Model file for the job. Use its own axes, mm. Coordinates: 2 decimals unless noted, no trailing zeros. Loops run counter-clockwise (first coordinate to the right, second up) from the corner with the lowest first, then second, coordinate; pieces in that order, holes last. Notation, with made-up numbers: M 33.25,14 L 79.25,14 A18 ccw 79.25,44 Z; hole C 74.5,34 d6. An arc over 180 degrees is marked long. One line per question, with ' | ' between items. Start each with the question number.
```python
from build123d import *

# Parameters (mm, degrees)
SKETCH_1_W                   = 20
SKETCH_1_H                   = 220
EXTRUDE_1_DEPTH              = 17.5
HOLE_WIZARD_M8_1_D           = 9
HOLE_WIZARD_M8_1_CBORE_D     = 15
HOLE_WIZARD_M8_1_CBORE_DEPTH = 8.6
HOLE_WIZARD_M8_1_2_D         = 6.8
HOLE_WIZARD_M8_1_2_DEPTH     = 19.75
HOLE_WIZARD_M8_1_2_TIP       = 2.042926105
CHAMFER_1_SIZE               = 1


with BuildPart() as part:
    # 草图1 → 凸台-拉伸1 (new, symmetric)
    with BuildSketch(Plane.XY):
        Rectangle(SKETCH_1_W, SKETCH_1_H)
    extrude(amount=EXTRUDE_1_DEPTH, both=True)

    # Hole Wizard M8 _1 (through all)
    with Locations(Plane.XY.offset(17.5)):
        with Locations((0, 100), (0, 0), (0, -100)):
            CounterBoreHole(HOLE_WIZARD_M8_1_D / 2, HOLE_WIZARD_M8_1_CBORE_D / 2, HOLE_WIZARD_M8_1_CBORE_DEPTH)

    # Hole Wizard M8 _1 2
    with Locations(Plane.XY.offset(17.5)):
        with Locations((0, 80), (0, -80)):
            Hole(HOLE_WIZARD_M8_1_2_D / 2, depth=HOLE_WIZARD_M8_1_2_DEPTH)
            with Locations((0, 0, -(HOLE_WIZARD_M8_1_2_DEPTH + HOLE_WIZARD_M8_1_2_TIP / 2))):  # 118° drill point
                Cone(0, HOLE_WIZARD_M8_1_2_D / 2, HOLE_WIZARD_M8_1_2_TIP, mode=Mode.SUBTRACT)

    # 倒角1
    chamfer_1_edges = [part.edges().sort_by_distance(p)[0] for p in [
        (10, -110, 0),
        (-10, -110, 0),
        (-10, 110, 0),
        (10, 110, 0),
    ]]
    chamfer(chamfer_1_edges, length=CHAMFER_1_SIZE)


solid = part.part
```
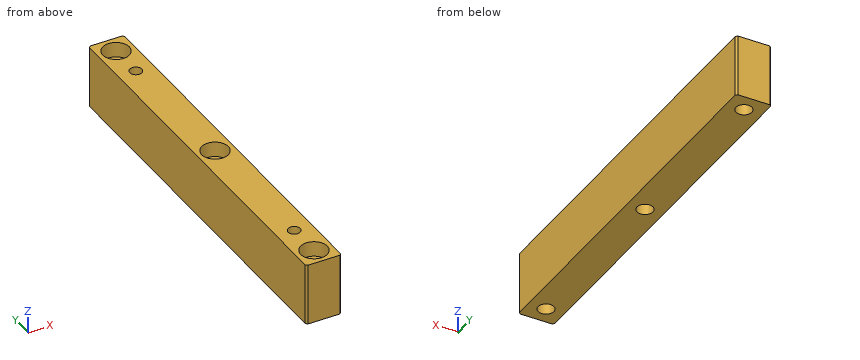
(1) Drill centre lines: line 1 (Y direction, x = 0, z = -9); line 2 (Y direction, x = 0, z = 10.5); line 3 (Y direction, x = 0, z = 5). Where is each one in solid material? Low to high. Write a range as [from, to].
(2) Band-saw the part on B-B on z = -7. Write the cut outline in (x, y).
(3) Band-saw the part on C-C on z = 2.5. Write the cut outline in (x, y).
(4) Pin check, flat tip, straight feed: P1, Ø4.5, axis at x = 2, y = 2.5, coming from the +Z side. Stop position of the tip, or through.
(5) Band-saw the part on A-A on y = 0. Write the cut outline in (x, z).
Computed values:
1) line 1: [-110, -104.5], [-95.5, -4.5], [4.5, 95.5], [104.5, 110] | line 2: [-110, -107.5], [-92.5, -83.4], [-76.6, -7.5], [7.5, 76.6], [83.4, 92.5], [107.5, 110] | line 3: [-110, -104.5], [-95.5, -83.4], [-76.6, -4.5], [4.5, 76.6], [83.4, 95.5], [104.5, 110]
2) outline: M -10,-109 L -9,-110 L 9,-110 L 10,-109 L 10,109 L 9,110 L -9,110 L -10,109 Z; hole C 0,-100 d9; hole C 0,0 d9; hole C 0,100 d9
3) outline: M -10,-109 L -9,-110 L 9,-110 L 10,-109 L 10,109 L 9,110 L -9,110 L -10,109 Z; hole C 0,-100 d9; hole C 0,0 d9; hole C 0,100 d9; hole C 0,-80 d6.8; hole C 0,80 d6.8
4) P1: z = 8.9
5) outline: M -10,-17.5 L -4.5,-17.5 L -4.5,8.9 L -7.5,8.9 L -7.5,17.5 L -10,17.5 Z; M 4.5,-17.5 L 10,-17.5 L 10,17.5 L 7.5,17.5 L 7.5,8.9 L 4.5,8.9 Z
